from build123d import *

# Parameters (mm, degrees)
BASE_PLATE_PROFILE_R        = 4
BASE_PLATE_PROFILE_W        = 1
BASE_PLATE_PROFILE_H        = 35
BASE_PLATE_PROFILE_W_2      = 24
BASE_PLATE_PROFILE_H_2      = 1
BASE_PLATE_PROFILE_H_3      = 34.5
BASE_PLATE_2MM_DEPTH        = 2
TAB_SEAT_RECESS_SKETCH_W    = 24
TAB_SEAT_RECESS_SKETCH_H    = 2
TAB_SEAT_RECESS_0_5MM_DEPTH = 0.5
SIDE_FLANGES_SKETCH_W       = 34.5
SIDE_FLANGES_SKETCH_H       = 2
SIDE_FLANGES_DEPTH          = 1
FLANGE_EXTENSION_DEPTH      = 1
REAR_TAB_SKETCH_W           = 24
REAR_TAB_SKETCH_H           = 20
REAR_TAB_24X20_DEPTH        = 1
REAR_TAB_CORNER_ROUND_R8_R  = 8
TAB_SLOT_DEPTH              = 2
TAB_ROOT_FILLET_R1_R        = 1
FLANGE_CROSS_HOLES_SKETCH_R = 2.5
FLANGE_CROSS_HOLES_DEPTH    = 50


with BuildPart() as part:
    # Base Plate Profile → Base Plate 2mm (new body)
    # profile 1 of 4: a face of its own
    with BuildSketch(Plane(origin=(0, 0, 0), x_dir=(1, 0, 0), z_dir=(0, 1, 0))):
        with BuildLine():
            Line((-13, 0), (-19, 0))
            Line((-19, 0), (-19, -35))
            Line((-19, -35), (-17, -35))
            Line((-17, -35), (-17, -36))
            Line((-17, -36), (-20, -36))
            Line((-20, -36), (-20, -40))
            Line((-20, -40), (-12.132851477, -59.380608198))
            ThreePointArc((-12.132851477, -59.380608198), (-10.292575783, -61.647471578), (-7.5, -62.5))
            Line((-7.5, -62.5), (7.5, -62.5))
            ThreePointArc((7.5, -62.5), (10.310807979, -61.63513706), (12.149230497, -59.339743401))
            Line((12.149230497, -59.339743401), (20, -39.5))
            Line((20, -39.5), (20, -35.5))
            Line((20, -35.5), (17, -35.5))
            Line((17, -35.5), (17, -34.5))
            Line((17, -34.5), (19, -34.5))
            Line((19, -34.5), (19, 0))
            Line((19, 0), (13, 0))
            Line((13, 0), (13, -3))
            Line((13, -3), (12, -3))
            Line((12, -3), (12, -0.5))
            Line((12, -0.5), (-12, -0.5))
            Line((-12, -0.5), (-12, -3))
            Line((-12, -3), (-13, -3))
            Line((-13, -3), (-13, 0))
        make_face()
        with Locations(Location((0, -49.5, 0), (0, 0, 270))):
            Circle(BASE_PLATE_PROFILE_R, mode=Mode.SUBTRACT)
        Polygon((8, -19.530894994), (3.97324415, -26.443650727), (-4.02675585, -26.412755733), (-8, -19.469105006), (-3.97324415, -12.556349273), (4.02675585, -12.587244267), align=None, mode=Mode.SUBTRACT)
    # profile 2 of 4: a face of its own
    with BuildSketch(Plane(origin=(0, 0, 0), x_dir=(1, 0, 0), z_dir=(0, 1, 0))):
        with Locations((-19.5, -17.5)):
            Rectangle(BASE_PLATE_PROFILE_W, BASE_PLATE_PROFILE_H)
    # profile 3 of 4: a face of its own
    with BuildSketch(Plane(origin=(0, 0, 0), x_dir=(1, 0, 0), z_dir=(0, 1, 0))):
        Rectangle(BASE_PLATE_PROFILE_W_2, BASE_PLATE_PROFILE_H_2)
    # profile 4 of 4: a face of its own
    with BuildSketch(Plane(origin=(0, 0, 0), x_dir=(1, 0, 0), z_dir=(0, 1, 0))):
        with Locations((19.5, -17.25)):
            Rectangle(BASE_PLATE_PROFILE_W, BASE_PLATE_PROFILE_H_3)
    extrude(amount=BASE_PLATE_2MM_DEPTH)

    # Tab Seat Recess Sketch → Tab Seat Recess 0.5mm (cut)
    with BuildSketch(Plane(origin=(0, 0, -0.5), x_dir=(-1, 0, 0), z_dir=(0, 0, -1))):
        with Locations((0, 1)):
            Rectangle(TAB_SEAT_RECESS_SKETCH_W, TAB_SEAT_RECESS_SKETCH_H)
    extrude(amount=-TAB_SEAT_RECESS_0_5MM_DEPTH, mode=Mode.SUBTRACT)

    # Side Flanges Sketch → Side Flanges (add)
    with BuildSketch(Plane(origin=(20, 0, 0), x_dir=(0, 0, -1), z_dir=(1, 0, 0))):
        Polygon((0, 15), (-29.5, 15), (-34.5, 10), (-34.5, 2), (0, 2), align=None)
        with Locations((-17.25, 1)):
            Rectangle(SIDE_FLANGES_SKETCH_W, SIDE_FLANGES_SKETCH_H)
    extrude(amount=-SIDE_FLANGES_DEPTH)

    # Flange Extension Sketch → Flange Extension (add)
    with BuildSketch(Plane.ZY.offset(20)):
        Polygon((0, 15), (0, 0), (35, 0), (35, 10), (30, 15), align=None)
    extrude(amount=-FLANGE_EXTENSION_DEPTH)

    # Rear Tab Sketch → Rear Tab 24x20 (add)
    with BuildSketch(Plane(origin=(0, 0, 0), x_dir=(-1, 0, 0), z_dir=(0, 0, -1))):
        with Locations((0, 10)):
            Rectangle(REAR_TAB_SKETCH_W, REAR_TAB_SKETCH_H)
    extrude(amount=-REAR_TAB_24X20_DEPTH)

    # Rear Tab Corner Round R8
    rear_tab_corner_round_r8_edges = [part.edges().sort_by_distance(p)[0] for p in [
        (12, 20, 0.5),
        (-12, 20, 0.5),
    ]]
    fillet(rear_tab_corner_round_r8_edges, radius=REAR_TAB_CORNER_ROUND_R8_R)

    # Tab Slot Sketch → Tab Slot (cut)
    with BuildSketch(Plane.XY.offset(1)):
        with BuildLine():
            Line((-3.998880062, 14), (3.998880062, 14))
            ThreePointArc((3.998880062, 14), (5.998880062, 12), (3.998880062, 10))
            Line((3.998880062, 10), (-3.998880062, 10))
            ThreePointArc((-3.998880062, 10), (-5.998880062, 12), (-3.998880062, 14))
        make_face()
    extrude(amount=-TAB_SLOT_DEPTH, mode=Mode.SUBTRACT)

    # Tab Root Fillet R1
    tab_root_fillet_r1_edges = [part.edges().sort_by_distance(p)[0] for p in [
        (0, 2, 1),
    ]]
    fillet(tab_root_fillet_r1_edges, radius=TAB_ROOT_FILLET_R1_R)

    # Flange Cross Holes Sketch → Flange Cross Holes (cut)
    with BuildSketch(Plane.ZY.offset(20)):
        with Locations((10, 8)):
            Circle(FLANGE_CROSS_HOLES_SKETCH_R)
        with Locations((25, 8)):
            Circle(FLANGE_CROSS_HOLES_SKETCH_R)
    extrude(amount=-FLANGE_CROSS_HOLES_DEPTH, mode=Mode.SUBTRACT)


solid = part.part
CAD build for the part. Positions are in the model's coordinates, mm. A direction names the side the tool comes from. Round coordinates to 2 decimals unless told otherwise and drop trailing zeros. Order: outer loops, then holes, each group sorted by start corner. A loop starts at its lowest first (then second) coordinate and runs counter-clockwise, first axis right, second up. Notation, with made-up numbers: (27, 35.5) -> (48, 35.5) arc R9 ccw to (48, 52.5) -> close; hole circle Ø3 at (51.25, -3.75). An arc over 180 degrees is marked (long way). Write item = value, one per line. Start each with the question number.
(1) Pin check, flat tips, straight feed: P1, Ø5, axis at x = 1, y = 13, coming from the +Z side; P2, Ø7, axis at x = 0, z = 49.5, coming from the -Y side; P3, Ø5, axis at x = 2, z = 31.5, coming from the +Y side; P4, Ø3.5, axis at x = 19, y = 4, coming from the +Z side. Stop position of each tip, or through.
(2) Cut at C-C, the plane x = 2. List the corners of the cut face in (y, z), then the cut area to 3 significant figures.
(3) Cut at B-B, the plane y = 8. List the corners of the cut face in (x, z).
(4) Which spindle directions (+Z, -Z, +X, -X, +Y, -Y) get a long thin tool onto all of the face, cutting with end or side? Do faces 1 (the cylindrical face through (-6, 12, 0.5)), 2 (the flat face through (19.2, 4, 34.5)), 3 (the flat face through (13, 1, 1)), 4 (the flat face through (0.2, 9.7, 1)), 5 (the flat face through (-18, 1, 36)). Say none if no direction does.
(5) Probe line 1 (Y direction, x = 19.7, z = 25); line 2 (X direction, y = 14, z = 5.5); line 3 (Y direction, x = -10, z = 58). List the from-to ranges inside material, lowest first. Write a range as [from, to].
(6) Pull direction Y, two halves, no side cores. Call faces 6 (the cylindrical face through (19.49, 5.56, 9.46)), 7 (the flat face through (-19.2, 3.8, 35)), 8 (the flat face through (0, 2, 31)): released by +Y, released by -Y, zero draft, split by the parting line, or undercut.
(7) Cut at D-D, the plane z = 25. List the corners of the cut face in (x, y).
(8) Cut at A-A, the plane z = 10. List the corners of the cut face in (x, y).
Model answer:
q1.P1 = 1
q1.P2 = through
q1.P3 = 2
q1.P4 = 34.5
q2.outline = (0, 0) -> (10, 0) -> (10, 1) -> (3, 1) arc R1 cw to (2, 2) -> (2, 12.58) -> (0, 12.58) -> close; (0, 26.44) -> (2, 26.44) -> (2, 46.04) -> (0, 46.04) -> close; (0, 52.96) -> (2, 52.96) -> (2, 62.5) -> (0, 62.5) -> close; (14, 0) -> (20, 0) -> (20, 1) -> (14, 1) -> close
q2.area = 97.6 mm2
q3.outline = (-20, 0) -> (-19, 0) -> (-19, 7.5) -> (-20, 7.5) -> close; (-20, 12.5) -> (-19, 12.5) -> (-19, 22.5) -> (-20, 22.5) -> close; (-20, 27.5) -> (-19, 27.5) -> (-19, 35) -> (-20, 35) -> close; (-12, 0) -> (12, 0) -> (12, 1) -> (-12, 1) -> close; (19, 0) -> (20, 0) -> (20, 7.5) -> (19, 7.5) -> close; (19, 12.5) -> (20, 12.5) -> (20, 22.5) -> (19, 22.5) -> close; (19, 27.5) -> (20, 27.5) -> (20, 34.5) -> (19, 34.5) -> close
q4.face_1 = +Z, -Z
q4.face_2 = +X, +Y, -Y
q4.face_3 = -Z, +Y, -Y
q4.face_4 = +Z, +Y
q4.face_5 = -X, +Y, -Y
q5.line_1 = [0, 5.5], [10.5, 15]
q5.line_2 = [-20, -19], [19, 20]
q5.line_3 = [0, 2]
q6.face_6 = undercut
q6.face_7 = zero draft
q6.face_8 = released by +Y
q7.outline = (-20, 0) -> (-4.84, 0) -> (-4.84, 2) -> (-19, 2) -> (-19, 5.5) -> (-20, 5.5) -> close; (-20, 10.5) -> (-19, 10.5) -> (-19, 15) -> (-20, 15) -> close; (4.81, 0) -> (20, 0) -> (20, 5.5) -> (19, 5.5) -> (19, 2) -> (4.81, 2) -> close; (19, 10.5) -> (20, 10.5) -> (20, 15) -> (19, 15) -> close
q8.outline = (-20, 0) -> (20, 0) -> (20, 5.5) -> (19, 5.5) -> (19, 2) -> (-19, 2) -> (-19, 5.5) -> (-20, 5.5) -> close; (-20, 10.5) -> (-19, 10.5) -> (-19, 15) -> (-20, 15) -> close; (19, 10.5) -> (20, 10.5) -> (20, 15) -> (19, 15) -> close
